Work out the finished part from the listing and answer in its coordinate system (mm). Coordinates: 2 decimals unless noted, no trailing zeros. Order: outer loops, then holes, each group sorted by start corner. A loop starts at its lowest first (then second) coordinate and runs counter-clockwise, first axis right, second up.
1. The part is cut by section D-D, the plane y = 19. Give the vertices of the cut face in (x, z), then the cut area to 3 significant figures.
2. The part is cut by section A-A, the plane x = 15. Give the vertices of the cut face in (y, z).
3. Find the intervals of material crossed by probe 1 along Y at (x, z) = (19, 2.3); probe 2 along X at (y, z) = (-17.5, 1.65); probe 3 along X at (y, z) = (10.5, 0.45), in increasing order.
4. The part is cut by section B-B, the plane z = 1.5. Give the vertices of the cut face in (x, y), then the cut area to 3 significant figures.
5. The part is cut by section C-C, the plane x = 4. Give the vertices of the cut face in (y, z), then the cut area to 3 significant figures.
6. Flat-ended cylindrical pins translate along their axes: pin 1 Ø1.2 at (x, z) = (2, 1) entering from +Y; pin 2 Ø1.5 at (y, z) = (-16.5, 1.5) entering from -X. Find the tip coordinate at first contact, or state that the pin passes through.
```python
from build123d import *

# Parameters (mm, degrees)
BOSS_EXTRUDE1_DEPTH = 3


with BuildPart() as part:
    # Sketch1 → Boss-Extrude1 (new body)
    with BuildSketch(Plane.XY):
        Polygon((3, -18.58433147), (0.680763745, -18.58433147), (0.680763745, -28.385118219), (3, -28.385118219), (3, -34.192991848), (36.923110286, -34.192991848), (36.923110286, 25), (4.847061595, 25), (4.847061595, 0), (20, 0), (20, -12.894618578), (3, -12.894618578), align=None)
    extrude(amount=BOSS_EXTRUDE1_DEPTH)


solid = part.part
```
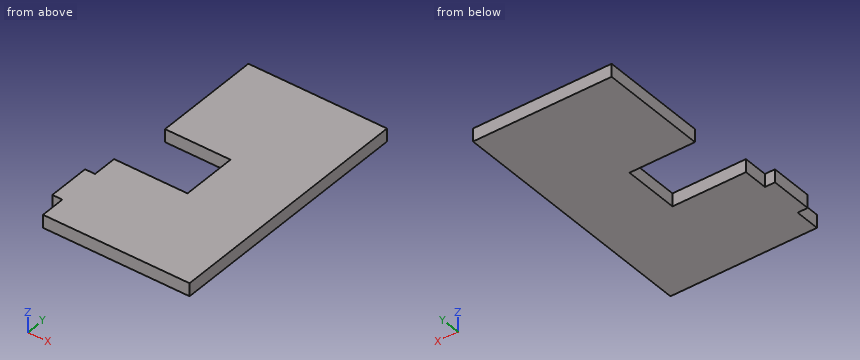
Geometry says:
1. outline: (4.85, 0) - (36.92, 0) - (36.92, 3) - (4.85, 3) - close
1. area: 96.2 mm2
2. outline: (-34.19, 0) - (-12.89, 0) - (-12.89, 3) - (-34.19, 3) - close; (0, 0) - (25, 0) - (25, 3) - (0, 3) - close
3. probe 1: y = -34.19 to -12.89, 0 to 25
3. probe 2: x = 3 to 36.92
3. probe 3: x = 4.85 to 36.92
4. outline: (0.68, -28.39) - (3, -28.39) - (3, -34.19) - (36.92, -34.19) - (36.92, 25) - (4.85, 25) - (4.85, 0) - (20, 0) - (20, -12.89) - (3, -12.89) - (3, -18.58) - (0.68, -18.58) - close
4. area: 1,770 mm2
5. outline: (-34.19, 0) - (-12.89, 0) - (-12.89, 3) - (-34.19, 3) - close
5. area: 63.9 mm2
6. pin 1: stops at y = -18.58
6. pin 2: stops at x = 3
